Can you work these out from the model? Positions are in its coordinate system, mm. A direction names the side the tool comes from. Round coordinates to 2 decimals unless told otherwise and drop trailing zeros. Write each loop counter-clockwise with the first axis right and the second up, starting at its lowest first coordinate (ties: lowest second). Pieces come first, ordered by that corner, then holes. Notation, with made-up numbers: M 12,49 L 30,49 A18 ccw 30,77 Z; hole C 40,58.25 d1. An arc over 180 degrees is marked long. Answer in a Markdown table with one row per item. Add a question column.
(1) If I drill on probe 1 along X at (y, z) = (12.7, 15.5); probe 2 along Y at (x, z) = (6.25, 64.5); probe 3 along X at (y, z) = (12.4, 58.5), over which ranges is the centre line in solid material (lowest first)?
(2) For faces 5 (the face through (-4.17, -12.51, 10.04)), 6 (the face through (-7.9, 12.5, 14.3)), 7 (the face through (0, 0, 0)), which set-ups out of +Z, -Z, +X, -X, +Y, -Y let a thin tool reach every point of the face, with its end or its side?
(3) Suppose I cut it at A-A, the plane z = 58.5. Write out the boundary of the cut face in (x, y).
(4) If we mould it in two halves opening along Z, with no side actions, what happens to faces 1 (the face through (0, -12, 29)), 2 (the face through (6.1, 12.5, 50.3)), 3 (the face through (13.5, 12, 24)), 4 (the face through (6.1, 12.5, 14.3))? For each: released by +Z, released by -Z, zero draft, split by the parting line, or undercut.
(5) Suppose I cut it at D-D, the plane x = -2.25. Write out the boundary of the cut face in (y, z), then the cut area to 3 significant figures.
(6) Suppose I cut it at C-C, the plane x = -10. Write out the boundary of the cut face in (y, z), then the cut area to 3 significant figures.
(7) Suppose I cut it at B-B, the plane z = 51.5. Write out the boundary of the cut face in (x, y), then the cut area to 3 significant figures.
(8) I'm going to push flat-ended pins straight in: pin 1 (2 mm diameter, centred on x = 8.5, y = -7.5, fed in from +Z); pin 2 (1.8 mm diameter, centred on x = -5.66, z = 21.16, fed in from -Y); pin 3 (1 mm diameter, centred on x = 4.5, y = -12.5, fed in from +Z). Where does each tip first touch, or does it pass through?
from build123d import *

# Parameters (mm, degrees)
SKETCH1_W           = 27
SKETCH1_H           = 27
BOSS_EXTRUDE1_DEPTH = 29
SKETCH2_W           = 27
SKETCH2_H           = 23
CUT_EXTRUDE1_DEPTH  = 27
CUT_EXTRUDE2_REACH  = 43.86
SKETCH4_R           = 4
SKETCH4_R_2         = 1.5
CUT_EXTRUDE3_REACH  = 43.86
SKETCH5_R           = 1.5
FILLET1_R           = 2
SKETCH6_W           = 27
SKETCH6_H           = 2
BOSS_EXTRUDE2_DEPTH = 38.5
SKETCH7_R           = 4
SKETCH7_R_2         = 1.5
CUT_EXTRUDE4_DEPTH  = 2


with BuildPart() as part:
    # Sketch1 → Boss-Extrude1 (new body)
    with BuildSketch(Plane.XY):
        Rectangle(SKETCH1_W, SKETCH1_H)
    extrude(amount=BOSS_EXTRUDE1_DEPTH)

    # Sketch2 → Cut-Extrude1 (cut)
    with BuildSketch(Plane(origin=(13.5, 0, 0), x_dir=(0, 0, -1), z_dir=(1, 0, 0))):
        with Locations((-15.5, 0)):
            Rectangle(SKETCH2_W, SKETCH2_H)
    extrude(amount=-CUT_EXTRUDE1_DEPTH, mode=Mode.SUBTRACT)

    # Sketch4 → Cut-Extrude2 (cut, up to next)
    with BuildSketch(Plane(origin=(0, 13.5, 0), x_dir=(1, 0, 0), z_dir=(0, 1, 0)), mode=Mode.PRIVATE) as cut_extrude2_sk1:
        with Locations(Location((0, -15.5, 0), (0, 0, 270))):
            Circle(SKETCH4_R)
    cut_extrude2_tool1 = extrude(cut_extrude2_sk1.sketch, amount=-CUT_EXTRUDE2_REACH, mode=Mode.PRIVATE) & part.part
    # Sketch4 → Cut-Extrude2 (cut, up to next)
    with BuildSketch(Plane(origin=(0, 13.5, 0), x_dir=(1, 0, 0), z_dir=(0, 1, 0)), mode=Mode.PRIVATE) as cut_extrude2_sk2:
        with Locations(Location((0, -8.5, 0), (0, 0, 270))):
            Circle(SKETCH4_R_2)
    cut_extrude2_tool2 = extrude(cut_extrude2_sk2.sketch, amount=-CUT_EXTRUDE2_REACH, mode=Mode.PRIVATE) & part.part
    # Sketch4 → Cut-Extrude2 (cut, up to next)
    with BuildSketch(Plane(origin=(0, 13.5, 0), x_dir=(1, 0, 0), z_dir=(0, 1, 0)), mode=Mode.PRIVATE) as cut_extrude2_sk3:
        with Locations(Location((7, -15.5, 0), (0, 0, 270))):
            Circle(SKETCH4_R_2)
    cut_extrude2_tool3 = extrude(cut_extrude2_sk3.sketch, amount=-CUT_EXTRUDE2_REACH, mode=Mode.PRIVATE) & part.part
    # Sketch4 → Cut-Extrude2 (cut, up to next)
    with BuildSketch(Plane(origin=(0, 13.5, 0), x_dir=(1, 0, 0), z_dir=(0, 1, 0)), mode=Mode.PRIVATE) as cut_extrude2_sk4:
        with Locations(Location((0, -22.5, 0), (0, 0, 270))):
            Circle(SKETCH4_R_2)
    cut_extrude2_tool4 = extrude(cut_extrude2_sk4.sketch, amount=-CUT_EXTRUDE2_REACH, mode=Mode.PRIVATE) & part.part
    # Sketch4 → Cut-Extrude2 (cut, up to next)
    with BuildSketch(Plane(origin=(0, 13.5, 0), x_dir=(1, 0, 0), z_dir=(0, 1, 0)), mode=Mode.PRIVATE) as cut_extrude2_sk5:
        with Locations(Location((-7, -15.5, 0), (0, 0, 270))):
            Circle(SKETCH4_R_2)
    cut_extrude2_tool5 = extrude(cut_extrude2_sk5.sketch, amount=-CUT_EXTRUDE2_REACH, mode=Mode.PRIVATE) & part.part
    add(cut_extrude2_tool1.solids().sort_by_distance((0, 13.5, 15.5))[0], mode=Mode.SUBTRACT)
    add(cut_extrude2_tool2.solids().sort_by_distance((0, 13.5, 8.5))[0], mode=Mode.SUBTRACT)
    add(cut_extrude2_tool3.solids().sort_by_distance((7, 13.5, 15.5))[0], mode=Mode.SUBTRACT)
    add(cut_extrude2_tool4.solids().sort_by_distance((0, 13.5, 22.5))[0], mode=Mode.SUBTRACT)
    add(cut_extrude2_tool5.solids().sort_by_distance((-7, 13.5, 15.5))[0], mode=Mode.SUBTRACT)

    # Sketch5 → Cut-Extrude3 (cut, up to next)
    with BuildSketch(Plane.XZ.offset(13.5), mode=Mode.PRIVATE) as cut_extrude3_sk1:
        with Locations(Location((0, 15.5, 0), (0, 0, 270))):
            Circle(SKETCH5_R)
    cut_extrude3_tool1 = extrude(cut_extrude3_sk1.sketch, amount=-CUT_EXTRUDE3_REACH, mode=Mode.PRIVATE) & part.part
    # Sketch5 → Cut-Extrude3 (cut, up to next)
    with BuildSketch(Plane.XZ.offset(13.5), mode=Mode.PRIVATE) as cut_extrude3_sk2:
        with Locations(Location((-5.656854249, 21.156854249, 0), (0, 0, 270))):
            Circle(SKETCH5_R)
    cut_extrude3_tool2 = extrude(cut_extrude3_sk2.sketch, amount=-CUT_EXTRUDE3_REACH, mode=Mode.PRIVATE) & part.part
    # Sketch5 → Cut-Extrude3 (cut, up to next)
    with BuildSketch(Plane.XZ.offset(13.5), mode=Mode.PRIVATE) as cut_extrude3_sk3:
        with Locations(Location((5.656854249, 21.156854249, 0), (0, 0, 270))):
            Circle(SKETCH5_R)
    cut_extrude3_tool3 = extrude(cut_extrude3_sk3.sketch, amount=-CUT_EXTRUDE3_REACH, mode=Mode.PRIVATE) & part.part
    # Sketch5 → Cut-Extrude3 (cut, up to next)
    with BuildSketch(Plane.XZ.offset(13.5), mode=Mode.PRIVATE) as cut_extrude3_sk4:
        with Locations(Location((5.656854249, 9.843145751, 0), (0, 0, 270))):
            Circle(SKETCH5_R)
    cut_extrude3_tool4 = extrude(cut_extrude3_sk4.sketch, amount=-CUT_EXTRUDE3_REACH, mode=Mode.PRIVATE) & part.part
    # Sketch5 → Cut-Extrude3 (cut, up to next)
    with BuildSketch(Plane.XZ.offset(13.5), mode=Mode.PRIVATE) as cut_extrude3_sk5:
        with Locations(Location((-5.656854249, 9.843145751, 0), (0, 0, 270))):
            Circle(SKETCH5_R)
    cut_extrude3_tool5 = extrude(cut_extrude3_sk5.sketch, amount=-CUT_EXTRUDE3_REACH, mode=Mode.PRIVATE) & part.part
    add(cut_extrude3_tool1.solids().sort_by_distance((0, -13.5, 15.5))[0], mode=Mode.SUBTRACT)
    add(cut_extrude3_tool2.solids().sort_by_distance((-5.656854, -13.5, 21.156854))[0], mode=Mode.SUBTRACT)
    add(cut_extrude3_tool3.solids().sort_by_distance((5.656854, -13.5, 21.156854))[0], mode=Mode.SUBTRACT)
    add(cut_extrude3_tool4.solids().sort_by_distance((5.656854, -13.5, 9.843146))[0], mode=Mode.SUBTRACT)
    add(cut_extrude3_tool5.solids().sort_by_distance((-5.656854, -13.5, 9.843146))[0], mode=Mode.SUBTRACT)

    # Fillet1
    fillet1_edges = [part.edges().sort_by_distance(p)[0] for p in [
        (0, -13.5, 0),
        (0, 13.5, 0),
    ]]
    fillet(fillet1_edges, radius=FILLET1_R)

    # Sketch6 → Boss-Extrude2 (add)
    with BuildSketch(Plane.XY.offset(29)):
        with Locations((0, 12.5)):
            Rectangle(SKETCH6_W, SKETCH6_H)
    extrude(amount=BOSS_EXTRUDE2_DEPTH)

    # Sketch7 → Cut-Extrude4 (cut)
    with BuildSketch(Plane(origin=(0, 13.5, 0), x_dir=(1, 0, 0), z_dir=(0, 1, 0))):
        with Locations(Location((0, -51.5, 0), (0, 0, 270))):
            Circle(SKETCH7_R)
        with Locations(Location((0, -44.5, 0), (0, 0, 270))):
            Circle(SKETCH7_R_2)
        with Locations(Location((7, -51.5, 0), (0, 0, 270))):
            Circle(SKETCH7_R_2)
        with Locations(Location((0, -58.5, 0), (0, 0, 270))):
            Circle(SKETCH7_R_2)
        with Locations(Location((-7, -51.5, 0), (0, 0, 270))):
            Circle(SKETCH7_R_2)
    extrude(amount=-CUT_EXTRUDE4_DEPTH, mode=Mode.SUBTRACT)


solid = part.part
Calculated:
| question | item | result |
|---|---|---|
| 1 | probe 1 | -13.5 to -8.5, -5.5 to -4, 4 to 5.5, 8.5 to 13.5 |
| 1 | probe 2 | 11.5 to 13.5 |
| 1 | probe 3 | -13.5 to -1.5, 1.5 to 13.5 |
| 2 | face 5 | -Y |
| 2 | face 6 | +Y |
| 2 | face 7 | -Z, +X, -X, +Y, -Y |
| 3 | outline | M -13.5,11.5 L -1.5,11.5 L -1.5,13.5 L -13.5,13.5 Z; M 1.5,11.5 L 13.5,11.5 L 13.5,13.5 L 1.5,13.5 Z |
| 4 | face 1 | released by +Z |
| 4 | face 2 | undercut |
| 4 | face 3 | zero draft |
| 4 | face 4 | undercut |
| 5 | outline | M -13.5,2 A2 ccw -11.5,0 L 11.5,0 A2 ccw 13.5,2 L 13.5,12.19 L 11.5,12.19 L 11.5,2 L -11.5,2 L -11.5,29 L -13.5,29 Z; M 11.5,18.81 L 13.5,18.81 L 13.5,48.19 L 11.5,48.19 Z; M 11.5,54.81 L 13.5,54.81 L 13.5,67.5 L 11.5,67.5 Z |
| 5 | area | 211 mm² |
| 6 | outline | M -13.5,2 A2 ccw -11.5,0 L 11.5,0 A2 ccw 13.5,2 L 13.5,67.5 L 11.5,67.5 L 11.5,2 L -11.5,2 L -11.5,29 L -13.5,29 Z |
| 6 | area | 237 mm² |
| 7 | outline | M -13.5,11.5 L -8.5,11.5 L -8.5,13.5 L -13.5,13.5 Z; M -5.5,11.5 L -4,11.5 L -4,13.5 L -5.5,13.5 Z; M 4,11.5 L 5.5,11.5 L 5.5,13.5 L 4,13.5 Z; M 8.5,11.5 L 13.5,11.5 L 13.5,13.5 L 8.5,13.5 Z |
| 7 | area | 26.0 mm² |
| 8 | pin 1 | z = 2 |
| 8 | pin 2 | y = 11.5 |
| 8 | pin 3 | z = 29 |
